Input: dimensioned drawing with shaded views. Units: mm. Origin: part minimum x, y, z. Give positions to 0.01 mm unless a question says otherwise; leave off trailing zeros. Write each loop counter-clockwise with the first axis right and the second up, starting at its lowest first coordinate (ties: lowest second). Pieces come first, ordered by that corner, then holes. Notation, with made-up numbers: (32, 76) - (60, 76) arc R36 ccw to (60, 115) - close; hole circle Ø3 at (56.25, -35.5). An arc over 180 degrees is marked (long way). Answer as a JSON object with one key per item and string values. Group by question number.
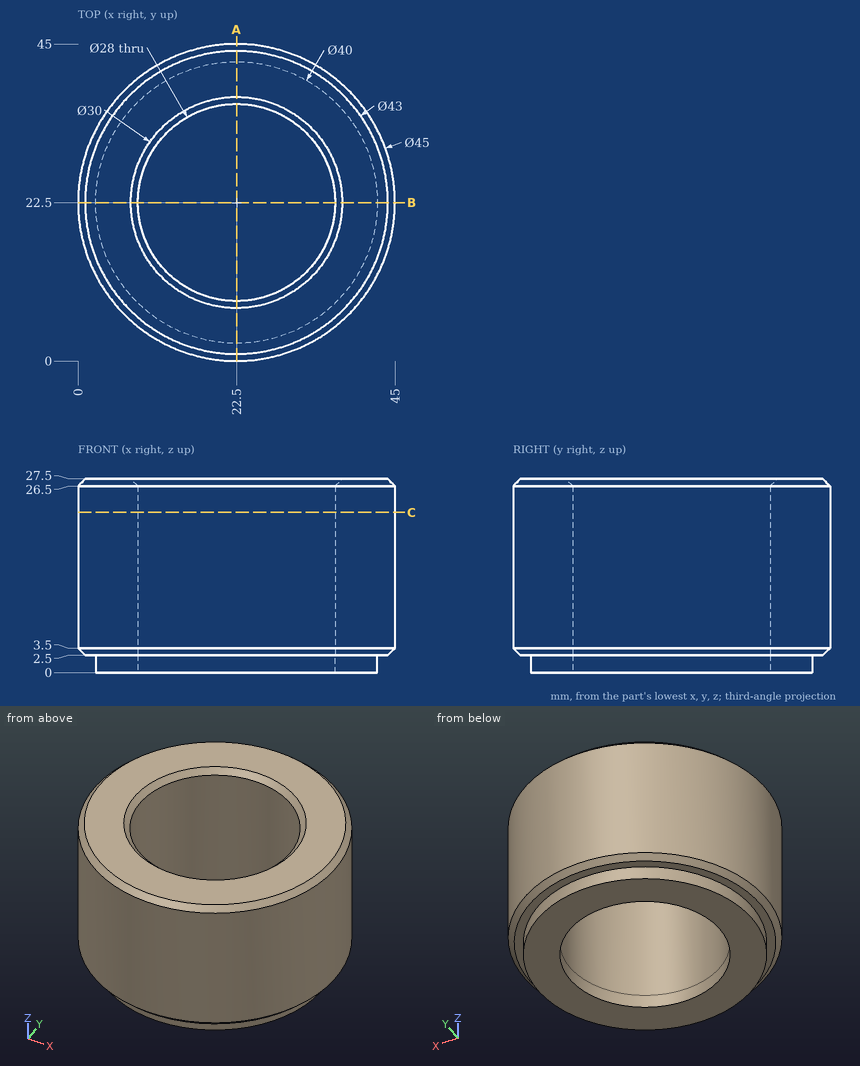
1) Cut plane C-C on z = 22.75. Return the cut outline in (x, y), and give its area (3 significant figures).
2) Line query: line 1 along Y through (x, z) = (22.5, 13); line 2 along X through (y, z) = (22, 5.5); line 3 along Y through (x, z) = (22.5, 0.6). Output: solid intervals per line, ascending. Write a range as from..to.
3) Pin query (flat end, axial travel): P1, Ø5, axis at y = 26.5, z = 14, coming from the +X side; P2, Ø8, axis at x = 17, y = 25, coming from the +Z side; P3, Ø1.5, axis at x = 17.5, z = 17.5, coming from the +Y side; P4, Ø12, axis at x = 8, z = 17.5, coming from the -Y side. Return the tip coordinate at first contact, or that it passes through.
4) Cut plane A-A on x = 22.5. Return the cut outline in (y, z).
Filled in:
{
 "1": {"outline": "circle Ø45 at (22.5, 22.5); hole circle Ø28 at (22.5, 22.5)", "area": "975 mm²"},
 "2": {"line 1": "y = 0..8.5, 36.5..45", "line 2": "x = 0.01..8.51, 36.49..44.99", "line 3": "y = 2.5..8.5, 36.5..42.5"},
 "3": {"P1": "stops at x = 44.95", "P2": "passes through", "P3": "stops at y = 44.59", "P4": "stops at y = 1.67"},
 "4": {"outline": "(0, 3.5) - (1, 2.5) - (2.5, 2.5) - (2.5, 0) - (8.5, 0) - (8.5, 26.5) - (7.5, 27.5) - (1, 27.5) - (0, 26.5) - close; (36.5, 0) - (42.5, 0) - (42.5, 2.5) - (44, 2.5) - (45, 3.5) - (45, 26.5) - (44, 27.5) - (37.5, 27.5) - (36.5, 26.5) - close"}
}
